Geometry: see drawing. Coordinates: mm, zero at the bounding-box minimum. Coordinates: 2 decimals unless noted, no trailing zeros. Loops run counter-clockwise (first coordinate to the right, second up) from the corner with the lowest first, then second, coordinate; pieces in that order, holes last. Notation, with made-up numbers: (-15, 76) -> (34, 76) arc R20 ccw to (34, 83) -> close; hole circle Ø1 at (0.5, 80). An arc over 180 degrees is marked (long way). One line per item, written item: value. Start each with the question number.
Item 1: Section query C-C on z = 2. Return loops of the section in (x, y).
Item 2: Ray query, probe 1 along Y at (x, z) = (42.5, 0.75); probe 2 along X at (y, z) = (10, 0.7); probe 3 along Y at (x, z) = (7.5, 1.55). Return the intervals inside material, ascending. Write a range as from..to.
Item 3: Mould query, pull axis X, two halves, no side actions, for the marked faces 1, 2 and 3. Classes: +X half, -X half, draft (parallel to the pull), parting line (faces both ways), or undercut.
Item 4: Section query B-B on y = 10. Return loops of the section in (x, z), then the cut area to 4 significant figures.
Item 5: Section query A-A on x = 42.5. Return loops of the section in (y, z), then the cut area to 3 significant figures.
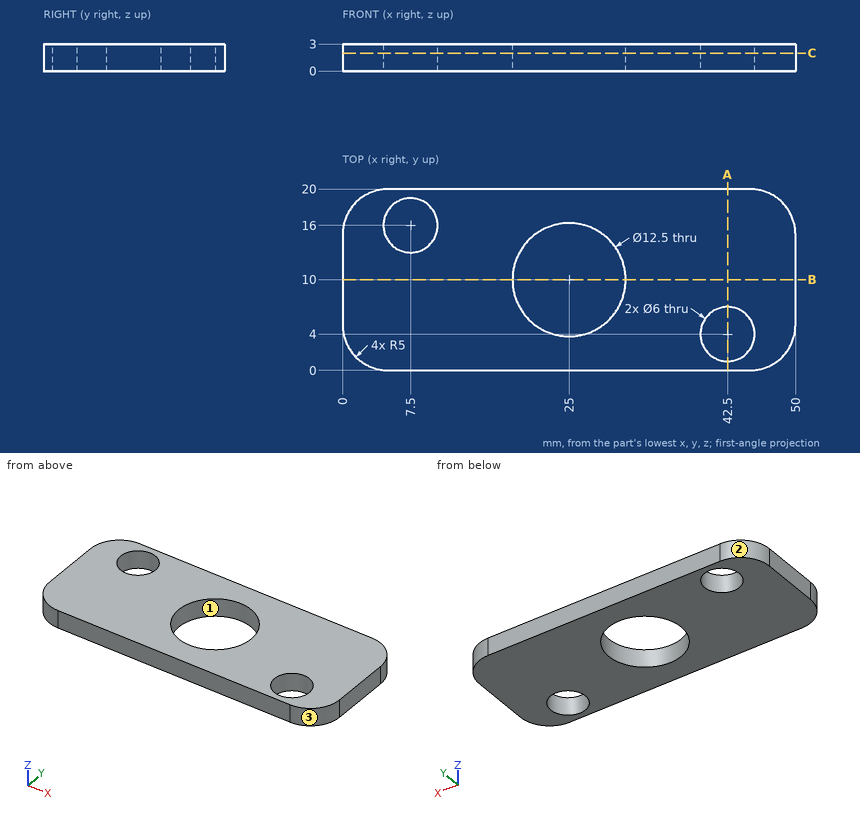
Reply:
1. outline: (0, 5) arc R5 ccw to (5, 0) -> (45, 0) arc R5 ccw to (50, 5) -> (50, 15) arc R5 ccw to (45, 20) -> (5, 20) arc R5 ccw to (0, 15) -> close; hole circle Ø6 at (7.5, 16); hole circle Ø12.5 at (25, 10); hole circle Ø6 at (42.5, 4)
2. probe 1: y = 0..1, 7..20
2. probe 2: x = 0..18.75, 31.25..50
2. probe 3: y = 0..13, 19..20
3. face 1: undercut
3. face 2: -X half
3. face 3: +X half
4. outline: (0, 0) -> (18.75, 0) -> (18.75, 3) -> (0, 3) -> close; (31.25, 0) -> (50, 0) -> (50, 3) -> (31.25, 3) -> close
4. area: 112.5 mm²
5. outline: (0, 0) -> (1, 0) -> (1, 3) -> (0, 3) -> close; (7, 0) -> (20, 0) -> (20, 3) -> (7, 3) -> close
5. area: 42.0 mm²
